from build123d import *

# Parameters (mm, degrees)
SKETCH1_W           = 21
SKETCH1_H           = 4
BOSS_EXTRUDE1_DEPTH = 10
SKETCH2_R           = 2
CUT_EXTRUDE1_DEPTH  = 10
CHAMFER2_SIZE       = 0.5


with BuildPart() as part:
    # Sketch1 → Boss-Extrude1 (new body)
    with BuildSketch(Plane.XY):
        with Locations((10.5, -2)):
            Rectangle(SKETCH1_W, SKETCH1_H)
    extrude(amount=BOSS_EXTRUDE1_DEPTH)

    # Sketch2 → Cut-Extrude1 (cut)
    with BuildSketch(Plane(origin=(0, 0, 0), x_dir=(1, 0, 0), z_dir=(0, 1, 0))):
        with Locations(Location((17, -5, 0), (0, 0, 270))):
            Circle(SKETCH2_R)
        with Locations(Location((4, -5, 0), (0, 0, 270))):
            Circle(SKETCH2_R)
    extrude(amount=-CUT_EXTRUDE1_DEPTH, mode=Mode.SUBTRACT)

    # Chamfer2
    chamfer2_edges = [part.edges().sort_by_distance(p)[0] for p in [
        (21, -2, 10),
        (0, -2, 10),
        (21, -2, 0),
        (10.5, -4, 0),
        (0, -2, 0),
        (10.5, -4, 10),
        (21, -4, 5),
        (0, -4, 5),
    ]]
    chamfer(chamfer2_edges, length=CHAMFER2_SIZE)


solid = part.part
Work out the finished part from the listing and answer in its coordinate system (mm). Give positions to 0.01 mm unless a question says otherwise; leave off trailing zeros. Order: outer loops, then holes, each group sorted by start corner. A loop starts at its lowest first (then second) coordinate and runs counter-clockwise, first axis right, second up. Notation, with made-up numbers: (81.25, -17.75) -> (99.25, -17.75) arc R24 ccw to (99.25, 4.25) -> close; hole circle Ø5 at (-31, 45). An arc over 180 degrees is marked (long way). Answer as a JSON object with one key per item and string values. Group by question number.
1. Section B-B on y = -3 is taken. Determine the outline of the cut face in (x, z).
2. The mould has two halves that part along X. Classify faces 1 (the cylindrical face through (19, -2, 5)), 2 (the flat face through (10, -2, 10)), 3 (the flat face through (0, -2, 5)): released by +X, released by -X, zero draft, split by the parting line, or undercut.
3. Section D-D on z = 4 is taken. Determine the outline of the cut face in (x, y), plus the area to 3 significant figures.
4. Consider line 1 along X through (y, z) = (-2.05, 5); line 2 along X through (y, z) = (-3.7, 5); line 3 along Z through (x, y) = (4.5, -1.3). Determine where each line is inside the solid, lowest interval first. Write a range as [from, to].
5. Section C-C on x = 17 is taken. Determine the outline of the cut face in (y, z), plus the area to 4 significant figures.
6. Section A-A on z = 5 is taken. Determine the outline of the cut face in (x, y), plus the area to 4 significant figures.
Result sheet:
{
 "1": {"outline": "(0, 0.5) -> (0.5, 0) -> (20.5, 0) -> (21, 0.5) -> (21, 9.5) -> (20.5, 10) -> (0.5, 10) -> (0, 9.5) -> close; hole circle Ø4 at (4, 5); hole circle Ø4 at (17, 5)"},
 "2": {"face 1": "undercut", "face 2": "zero draft", "face 3": "released by -X"},
 "3": {"outline": "(0, -3.5) -> (0.5, -4) -> (2.27, -4) -> (2.27, 0) -> (0, 0) -> close; (5.73, -4) -> (15.27, -4) -> (15.27, 0) -> (5.73, 0) -> close; (18.73, -4) -> (20.5, -4) -> (21, -3.5) -> (21, 0) -> (18.73, 0) -> close", "area": "56.0 mm^2"},
 "4": {"line 1": "x = [0, 2], [6, 15], [19, 21]", "line 2": "x = [0.2, 2], [6, 15], [19, 20.8]", "line 3": "z = [0, 3.06], [6.94, 10]"},
 "5": {"outline": "(-4, 0.5) -> (-3.5, 0) -> (0, 0) -> (0, 3) -> (-4, 3) -> close; (-4, 7) -> (0, 7) -> (0, 10) -> (-3.5, 10) -> (-4, 9.5) -> close", "area": "23.75 mm^2"},
 "6": {"outline": "(0, -3.5) -> (0.5, -4) -> (2, -4) -> (2, 0) -> (0, 0) -> close; (6, -4) -> (15, -4) -> (15, 0) -> (6, 0) -> close; (19, -4) -> (20.5, -4) -> (21, -3.5) -> (21, 0) -> (19, 0) -> close", "area": "51.75 mm^2"}
}
